For this review, use the dimensioned drawing (mm, ordinates from the lowest corner) and the shaded views. A direction names the side the tool comes from. Round coordinates to 2 decimals unless told otherwise and drop trailing zeros. Write each loop counter-clockwise with the first axis right and the second up, starting at its lowest first coordinate (ties: lowest second). Pieces come first, ordered by that corner, then holes.
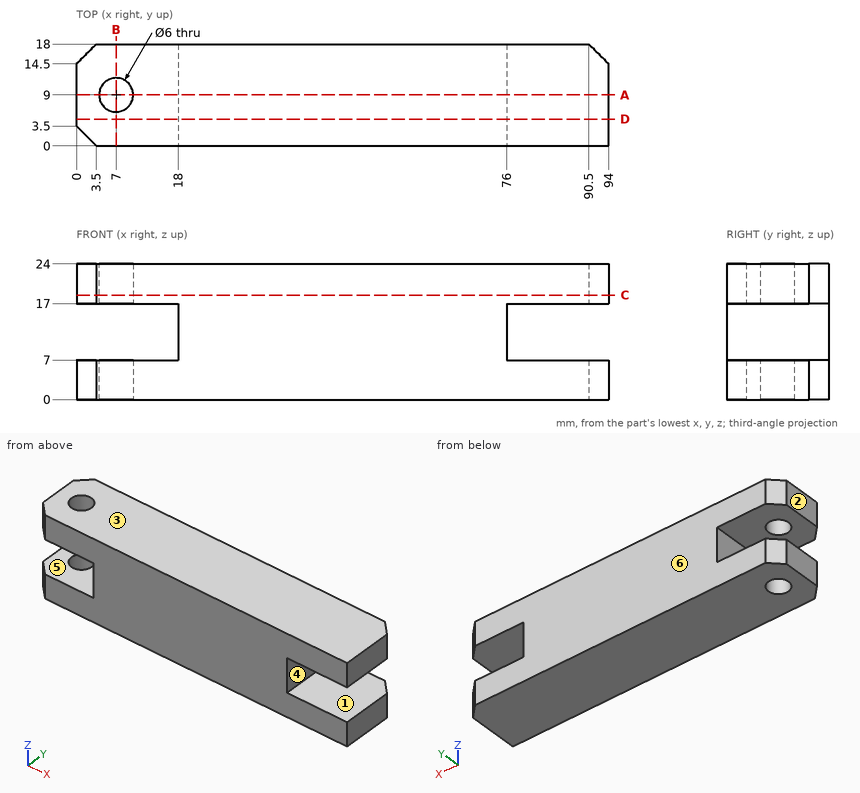
1) Add section A-A on y = 9. State the section outline as (x, z) points, and give its area (3 significant figures).
2) For the marked faces 4, 5 and 6, list the 3-axis set-ups (+Z, -Z, +X, -X, +Y, -Y) from which the entire face can be reached by the end or side of a thin tool; tool diameter is ignored.
3) The part is to be moulded in two halves that separate along Z. For the marked faces 1, 2 and 3, say which applies: pulls with the +Z half, pulls with the -Z half, needs draft (parallel to the pull), parting line crosses it, or undercut.
4) Add section C-C on z = 18.5. State the section outline as (x, y) points, and give its area (3 significant figures).
5) Add section B-B on x = 7. State the section outline as (y, z) points, and give its area (3 significant figures).
6) For line 1 along Y through (x, z) = (7, 21.5); line 2 along Z through (x, y) = (12.5, 6.5); line 3 along X through (y, z) = (5.5, 16.5), list the stretches that pass through material, from the lowest coordinate up.
7) Add section D-D on y = 4.75. State the section outline as (x, z) points.
Computed:
1. outline: (0, 0) - (4, 0) - (4, 7) - (0, 7) - close; (0, 17) - (4, 17) - (4, 24) - (0, 24) - close; (10, 0) - (94, 0) - (94, 7) - (76, 7) - (76, 17) - (94, 17) - (94, 24) - (10, 24) - (10, 17) - (18, 17) - (18, 7) - (10, 7) - close
1. area: 1,810 mm2
2. face 4: +X, +Y, -Y
2. face 5: -X, +Y, -Y
2. face 6: +Z, -Z, +X, -X, +Y
3. face 1: undercut
3. face 2: needs draft
3. face 3: pulls with the +Z half
4. outline: (0, 3.5) - (3.5, 0) - (94, 0) - (94, 14.5) - (90.5, 18) - (3.5, 18) - (0, 14.5) - close; hole circle Ø6 at (7, 9)
4. area: 1,650 mm2
5. outline: (0, 0) - (6, 0) - (6, 7) - (0, 7) - close; (0, 17) - (6, 17) - (6, 24) - (0, 24) - close; (12, 0) - (18, 0) - (18, 7) - (12, 7) - close; (12, 17) - (18, 17) - (18, 24) - (12, 24) - close
5. area: 168 mm2
6. line 1: y = 0 to 6, 12 to 18
6. line 2: z = 0 to 7, 17 to 24
6. line 3: x = 18 to 76
7. outline: (0, 0) - (94, 0) - (94, 7) - (76, 7) - (76, 17) - (94, 17) - (94, 24) - (0, 24) - (0, 17) - (18, 17) - (18, 7) - (0, 7) - close
